Design review of the part built by this model. Coordinates are the model's own, in mm. Face numbers are marked on the shaded views. A direction names the side the tool comes from. Coordinates: 2 decimals unless noted, no trailing zeros. Write each loop counter-clockwise with the first axis right and the second up, starting at its lowest first coordinate (ties: lowest second). Pieces come first, ordered by that corner, then holes. Notation, with made-up numbers: (-8, 71) - (7, 71) arc R17 ccw to (7, 75) - close; hole circle Ø1 at (83.5, -4.75). An arc over 180 degrees is marked (long way). Answer as a JSON object with one key per item and string values.
```python
from build123d import *

# Parameters (mm, degrees)
EXTRUDE_1_DEPTH           = 50
CHAMFER_1_SIZE            = 3
CUT_EXTRUDE_1_REACH       = 138.711
SKETCH_3_R                = 35.5
HOLE_WIZARD_1_D           = 6.6
HOLE_WIZARD_1_CBORE_D     = 11
HOLE_WIZARD_1_CBORE_DEPTH = 35


with BuildPart() as part:
    # 草图2 → 凸台-拉伸1 (new, symmetric)
    with BuildSketch(Plane(origin=(409.637600706, 0.5, -34.379468655), x_dir=(1, 0, 0), z_dir=(0, 0, 1))):
        Polygon((-409.637600706, 100.5), (-409.637600706, -0.5), (-454.637600706, -0.5), (-454.637600706, 15.5), (-417.637600706, 15.5), (-417.637600706, 100.5), align=None)
    extrude(amount=EXTRUDE_1_DEPTH, both=True)

    # 倒角1
    chamfer_1_edges = [part.edges().sort_by_distance(p)[0] for p in [
        (-45, 8, 15.620531345),
        (-4, 101, 15.620531345),
        (-45, 8, -84.379468655),
        (-4, 101, -84.379468655),
    ]]
    chamfer(chamfer_1_edges, length=CHAMFER_1_SIZE)

    # 草图3 → 切除-拉伸1 (cut, up to next)
    with BuildSketch(Plane.ZY.offset(8), mode=Mode.PRIVATE) as cut_extrude_1_sk1:
        with Locations((-34.379468655, 59)):
            Circle(SKETCH_3_R)
    cut_extrude_1_tool1 = extrude(cut_extrude_1_sk1.sketch, amount=-CUT_EXTRUDE_1_REACH, mode=Mode.PRIVATE) & part.part
    add(cut_extrude_1_tool1.solids().sort_by_distance((-8, 59, -34.379469))[0], mode=Mode.SUBTRACT)

    # 打孔尺寸(%根据)内六角圆柱头螺钉的类型1 (through all)
    with Locations(Plane(origin=(0, 8, 3.620531345), x_dir=(0, 0, 1), z_dir=(1, 0, 0))):
        with Locations((0, 0), (-38, 0), (-76, 0)):
            CounterBoreHole(HOLE_WIZARD_1_D / 2, HOLE_WIZARD_1_CBORE_D / 2, HOLE_WIZARD_1_CBORE_DEPTH)


solid = part.part
```
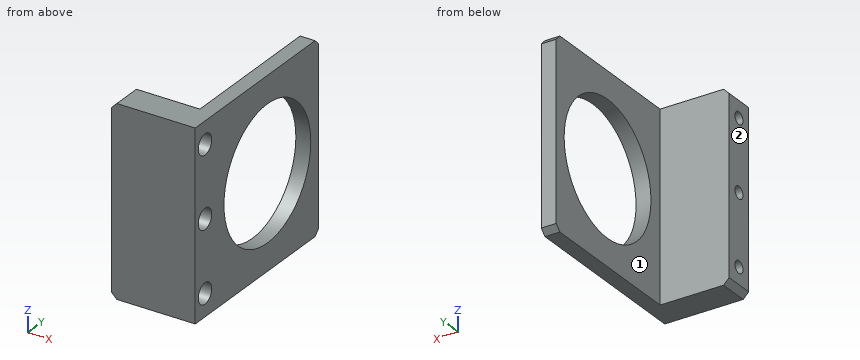
(1) Tool access review of the marked faces 1 and 2: name each direction out of +Z, -Z, +X, -X, +Y, -Y from which nothing blocks a thin tool from reaching the whole face with its end or side.
Solved:
{"face 1": "+Z, -Z, -X, +Y", "face 2": "+Z, -Z, -X, +Y, -Y"}
(2) Take a section at D-D, the plane z = -21.5. Write out the cut boundary in (x, y), and give its area (3 significant figures).
Solved:
{"outline": "(-45, 0) - (0, 0) - (0, 25.92) - (-8, 25.92) - (-8, 16) - (-45, 16) - close; (-8, 92.08) - (0, 92.08) - (0, 101) - (-8, 101) - close", "area": "871 mm^2"}
(3) Take a section at A-A, the plane y = 59. Write out the cut boundary in (x, z).
Solved:
{"outline": "(-8, -84.38) - (0, -84.38) - (0, -69.88) - (-8, -69.88) - close; (-8, 1.12) - (0, 1.12) - (0, 15.62) - (-8, 15.62) - close"}
(4) Take a section at C-C, the plane x = -14. Write out the cut boundary in (y, z), and give its area (3 significant figures).
Solved:
{"outline": "(0, -84.38) - (16, -84.38) - (16, 15.62) - (0, 15.62) - close; hole circle Ø11 at (8, -72.38); hole circle Ø11 at (8, -34.38); hole circle Ø11 at (8, 3.62)", "area": "1,310 mm^2"}
(5) Take a section at B-B, the plane y = 8. Give the number of separate pieces and of enclosed holes in the cut face, and give its area (3 significant figures).
Solved:
{"separate pieces": "4", "enclosed holes": "0", "area": "3,140 mm^2"}
(6) To check wall thickness, follow line 1 (Z direction, x = -41, y = 8); line 2 (Z direction, x = -6, y = 59.5); line 3 (Y direction, x = -33.5, z = -34). State the ranges of each line that lie inside material, in increasing order. Write a range as from..to.
Solved:
{"line 1": "z = -84.38..-75.68, -69.08..-37.68, -31.08..0.32, 6.92..15.62", "line 2": "z = -84.38..-69.88, 1.12..15.62", "line 3": "y = 0..2.51, 13.49..16"}
(7) For pin 1 (8 mm diameter, centred on y = 77.5, z = -59, fed in from +X); pin 2 (3.5 mm diameter, centred on y = 8.5, z = -32, fed in from +X); pin 3 (11 mm diameter, centred on x = -29.5, z = -36, fed in from +Y), all flat-tipped, find the tip position at first contact; note any pin that passes through.
Solved:
{"pin 1": "passes through", "pin 2": "stops at x = -35", "pin 3": "stops at y = 16"}
